```python
from build123d import *

# Parameters (mm, degrees)
SKETCH_1_W          = 270
SKETCH_1_H          = 30
EXTRUDE_1_DEPTH     = 40
SKETCH_2_R          = 10
CUT_EXTRUDE_2_DEPTH = 30
SKETCH_3_W          = 30
SKETCH_3_H          = 40
EXTRUDE_2_DEPTH     = 15
CUT_EXTRUDE_3_DEPTH = 159.113883008


with BuildPart() as part:
    # 草图1 → 凸台-拉伸1 (new body)
    with BuildSketch(Plane(origin=(0, 0, 0), x_dir=(1, 0, 0), z_dir=(0, 1, 0))):
        Rectangle(SKETCH_1_W, SKETCH_1_H)
    extrude(amount=EXTRUDE_1_DEPTH)

    # 草图2 → 切除-拉伸2 (cut)
    with BuildSketch(Plane(origin=(0, 40, 0), x_dir=(1, 0, 0), z_dir=(0, 1, 0))):
        with Locations(Location((70, 0, 0), (0, 0, 270))):
            Circle(SKETCH_2_R)
        with Locations(Location((-70, 0, 0), (0, 0, 90))):
            Circle(SKETCH_2_R)
    extrude(amount=-CUT_EXTRUDE_2_DEPTH, mode=Mode.SUBTRACT)

    # 草图3 → 凸台-拉伸2 (add)
    with BuildSketch(Plane.ZY.offset(135)):
        with Locations((0, 20)):
            Rectangle(SKETCH_3_W, SKETCH_3_H)
    extrude(amount=EXTRUDE_2_DEPTH)

    # 草图4 → 切除-拉伸3 (cut, through all)
    with BuildSketch(Plane.XY.offset(15)):
        Polygon((-150, 0), (-110, 40), (-150, 40), align=None)
    extrude(amount=-CUT_EXTRUDE_3_DEPTH, mode=Mode.SUBTRACT)


solid = part.part
```
Read the model definition and answer for the solid it produces. Units are mm, in the model's axes. A direction names the side the tool comes from. Round coordinates to 2 decimals unless told otherwise and drop trailing zeros. Write each loop counter-clockwise with the first axis right and the second up, starting at its lowest first coordinate (ties: lowest second). Pieces come first, ordered by that corner, then holes. Notation, with made-up numbers: M 88.25,62.5 L 94.25,62.5 A23 cw 94.25,74.5 Z; hole C -25,-1.75 d4. An arc over 180 degrees is marked long. One line per item, written item: value.
Q1. Find section D-D on y = 7.5. Write down the section's boundary in (x, z), plus the area to 4 significant figures.
Data:
outline: M -142.5,-15 L 135,-15 L 135,15 L -142.5,15 Z
area: 8,325 mm2
Q2. Which of the six approach directions +Z, -Z, +X, -X, +Y, -Y give full straight-line access (tool end or side, diameter ignored) to faces 1 (the flat face through (14, 40, 0)), 2 (the cylindrical face through (-79.915, 25.21, 1.302))?
Data:
face 1: +Z, -Z, +X, -X, +Y
face 2: +Y
Q3. Find section A-A on y = 22. Write down the section's boundary in (x, z).
Data:
outline: M -128,-15 L 135,-15 L 135,15 L -128,15 Z; hole C -70,0 d20; hole C 70,0 d20
Q4. Find section C-C on x = -70. Write down the section's boundary in (y, z), plus the area to 3 significant figures.
Data:
outline: M 0,-15 L 40,-15 L 40,-10 L 10,-10 L 10,10 L 40,10 L 40,15 L 0,15 Z
area: 600 mm2
Q5. For a pull along Z with two mould halves and no side action, classify faces 3 (the flat face through (-6, 20, -15)), 4 (the flat face through (-130, 20, 0)), 5 (the flat face through (-6, 20, 15)), 6 (the cylindrical face through (79.915, 25.21, -1.302)) as +Z half, -Z half, draft (parallel to the pull), parting line (faces both ways), or undercut.
Data:
face 3: -Z half
face 4: draft
face 5: +Z half
face 6: undercut
Q6. Find section B-B on z = 0. Write down the section's boundary in (x, y), plus the area to 3 significant figures.
Data:
outline: M -150,0 L 135,0 L 135,40 L 80,40 L 80,10 L 60,10 L 60,40 L -60,40 L -60,10 L -80,10 L -80,40 L -110,40 Z
area: 9,400 mm2
Q7. Straight lines are drawn through the part: line 1 (X direction, y = 20, z = 0); line 2 (X direction, y = 28.5, z = 0); line 3 (Z direction, x = -70, y = 30.25). For each, find the intervals that lie inside material, in ascending order. Write a range as [from, to].
Data:
line 1: [-130, -80], [-60, 60], [80, 135]
line 2: [-121.5, -80], [-60, 60], [80, 135]
line 3: [-15, -10], [10, 15]
Q8. Flat-ended cylindrical pins translate along their axes: pin 1 Ø12 at (x, z) = (70, 0) entering from +Y; pin 2 Ø3 at (y, z) = (21, 1.5) entering from -X; pin 3 Ø2 at (y, z) = (22.5, -1.5) entering from -X. Find the tip coordinate at first contact, or state that the pin passes through.
Data:
pin 1: y = 10
pin 2: x = -130.5
pin 3: x = -128.5
